```python
from build123d import *

# Parameters (mm, degrees)
SKETCH3_R           = 5
BOSS_EXTRUDE1_DEPTH = 10


with BuildPart() as part:
    # Sketch3 → Boss-Extrude1 (new body)
    with BuildSketch(Plane.XY):
        with BuildLine():
            Line((-15, 796.465754902), (70, -19.802144846))
            ThreePointArc((70, -19.802144846), (86.561987186, -33.24015766), (100, -16.678170473))
            Line((100, -16.678170473), (15, 799.589729274))
            ThreePointArc((15, 799.589729274), (-1.561987186, 813.027742088), (-15, 796.465754902))
        make_face()
        with Locations((0, 798.027742088)):
            Circle(SKETCH3_R, mode=Mode.SUBTRACT)
        with Locations((85, -18.24015766)):
            Circle(SKETCH3_R, mode=Mode.SUBTRACT)
    extrude(amount=BOSS_EXTRUDE1_DEPTH)


solid = part.part
```
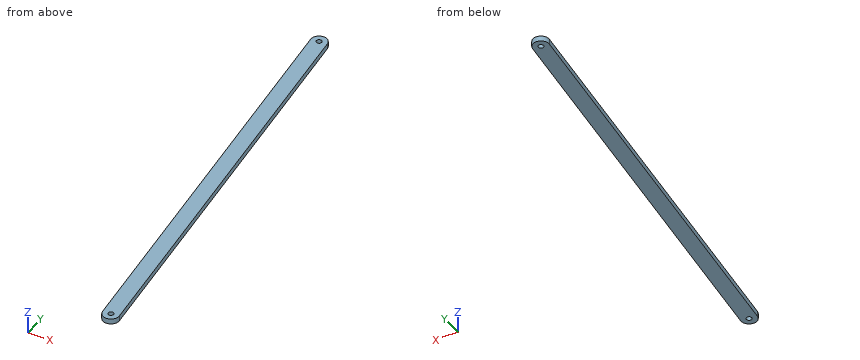
For this review, take the finished solid that the model builds, in its own axes (mm). Round coordinates to 2 decimals unless told otherwise and drop trailing zeros. Write each loop counter-clockwise with the first axis right and the second up, starting at its lowest first coordinate (ties: lowest second). Pieces come first, ordered by that corner, then holes. Notation, with made-up numbers: (-34.75, 70.5) - (14.25, 70.5) arc R6 ccw to (14.25, 79.5) - close; hole circle Ø11 at (29.5, 13.5). An arc over 180 degrees is marked (long way). Use CSV: the item, a comma, the result in double quotes.
1) Add section B-B on y = 262. Write out the cut boundary in (x, z), and give its area (3 significant figures).
Conclusion:
outline,"(40.66, 0) - (70.98, 0) - (70.98, 10) - (40.66, 10) - close"
area,"303 mm^2"
2) Add section C-C on x = 63. Write out the cut boundary in (y, z).
Conclusion:
outline,"(47.42, 0) - (338.64, 0) - (338.64, 10) - (47.42, 10) - close"
3) Wall thickness on line 1 along X through (y, z) = (334, 7.75); line 2 along X through (y, z) = (60, 5.75): over which ranges is each line inside the solid? List them lowest first. Write a range as from..to.
Conclusion:
line 1,"x = 33.16..63.48"
line 2,"x = 61.69..92.02"
4) Clearance check with flat-ended pins moving along their axes: pin 1 Ø4 at (y, z) = (197, 8.5) entering from +X; pin 2 Ø3 at (y, z) = (437.5, 5.5) entering from +X; pin 3 Ø1 at (x, z) = (81.5, 2) entering from -Y; pin 4 Ø6 at (x, y) = (85, -18.24) entering from +Z. State where each tip first meets the part, or that it passes through.
Conclusion:
pin 1,"stops at x = 77.96"
pin 2,"stops at x = 52.86"
pin 3,"stops at y = -33.02"
pin 4,"passes through"
5) Add section A-A on z = 7.5. Write out the cut boundary in (x, y).
Conclusion:
outline,"(-15, 796.47) - (70, -19.8) arc R15.08 ccw to (100, -16.68) - (15, 799.59) arc R15.08 ccw to start; hole circle Ø10 at (0, 798.03); hole circle Ø10 at (85, -18.24)"
